```python
from build123d import *

# Parameters (mm, degrees)
BOSS_EXTRUDE2_DEPTH = 337.5
SHELL1_T            = -6


with BuildPart() as part:
    # Sketch2 → Boss-Extrude2 (new body)
    with BuildSketch(Plane.XY):
        with BuildLine():
            Line((42, 25), (-42, 25))
            ThreePointArc((-42, 25), (-47.656854249, 22.656854249), (-50, 17))
            Line((-50, 17), (-50, -17))
            ThreePointArc((-50, -17), (-47.656854249, -22.656854249), (-42, -25))
            Line((-42, -25), (42, -25))
            ThreePointArc((42, -25), (47.656854249, -22.656854249), (50, -17))
            Line((50, -17), (50, 17))
            ThreePointArc((50, 17), (47.656854249, 22.656854249), (42, 25))
        make_face()
    extrude(amount=BOSS_EXTRUDE2_DEPTH)

    # Shell1
    shell1_openings = [part.faces().sort_by_distance(p)[0] for p in [
        (0, 0, 337.5),
        (0, 0, 0),
    ]]
    offset(amount=SHELL1_T, openings=shell1_openings, kind=Kind.INTERSECTION)


solid = part.part
```
Part model, mm, in its own coordinate system. A direction names the side the tool comes from. Round coordinates to 2 decimals unless told otherwise and drop trailing zeros. Write each loop counter-clockwise with the first axis right and the second up, starting at its lowest first coordinate (ties: lowest second). Pieces come first, ordered by that corner, then holes.
Item 1: Cut at C-C, the plane x = -15. Give the cut face in (y, z), plus the area to 3 significant figures.
Results:
outline: (-25, 0) - (-19, 0) - (-19, 337.5) - (-25, 337.5) - close; (19, 0) - (25, 0) - (25, 337.5) - (19, 337.5) - close
area: 4,050 mm2
Item 2: Probe L1, parallel to X at y = 14, z = 145; L2, parallel to Y at x = -31, z = 152; L3, parallel to Y at x = 43, z = 136. List the from-to ranges inside material, lowest first.
Results:
L1: x = -50 to -44, 44 to 50
L2: y = -25 to -19, 19 to 25
L3: y = -24.94 to -18.73, 18.73 to 24.94
Item 3: Which spindle directions (+Z, -Z, +X, -X, +Y, -Y) get a long thin tool onto all of the face, cutting with end or side? Do faces 1 (the cylindrical face through (47.719, 22.594, 166.388)), 2 (the flat face through (1, 19, 166)). Say none if no direction does.
Results:
face 1: +Z, -Z, +X, +Y
face 2: +Z, -Z
Item 4: Cut at A-A, the plane y = -2. Give the cut face in (x, z).
Results:
outline: (-50, 0) - (-44, 0) - (-44, 337.5) - (-50, 337.5) - close; (44, 0) - (50, 0) - (50, 337.5) - (44, 337.5) - close
Item 5: Drop a flat-ended pin along its axis: pin 1 Ø2 at (y, z) = (-18.5, 200.5) entering from -X. Give the stop position or say it passes through.
Results:
pin 1: stops at x = -49.98
Item 6: Cut at B-B, the plane z = 198. Give the cut face in (x, y).
Results:
outline: (-50, -17) arc R8 ccw to (-42, -25) - (42, -25) arc R8 ccw to (50, -17) - (50, 17) arc R8 ccw to (42, 25) - (-42, 25) arc R8 ccw to (-50, 17) - close; hole (-44, -17) arc R2 ccw to (-42, -19) - (42, -19) arc R2 ccw to (44, -17) - (44, 17) arc R2 ccw to (42, 19) - (-42, 19) arc R2 ccw to (-44, 17) - close
Item 7: Two-plate mould, pull along Y, no slides. Class faces 3 (the flat face through (-50, 0, 166)), 4 (the cylindrical face through (-47.594, 22.719, 166.388)), 5 (the flat face through (-44, 0, 166)), 6 (the flat face through (44, 0, 166)): +Y half, -Y half, draft (parallel to the pull), parting line (faces both ways), or undercut.
Results:
face 3: draft
face 4: +Y half
face 5: undercut
face 6: undercut
